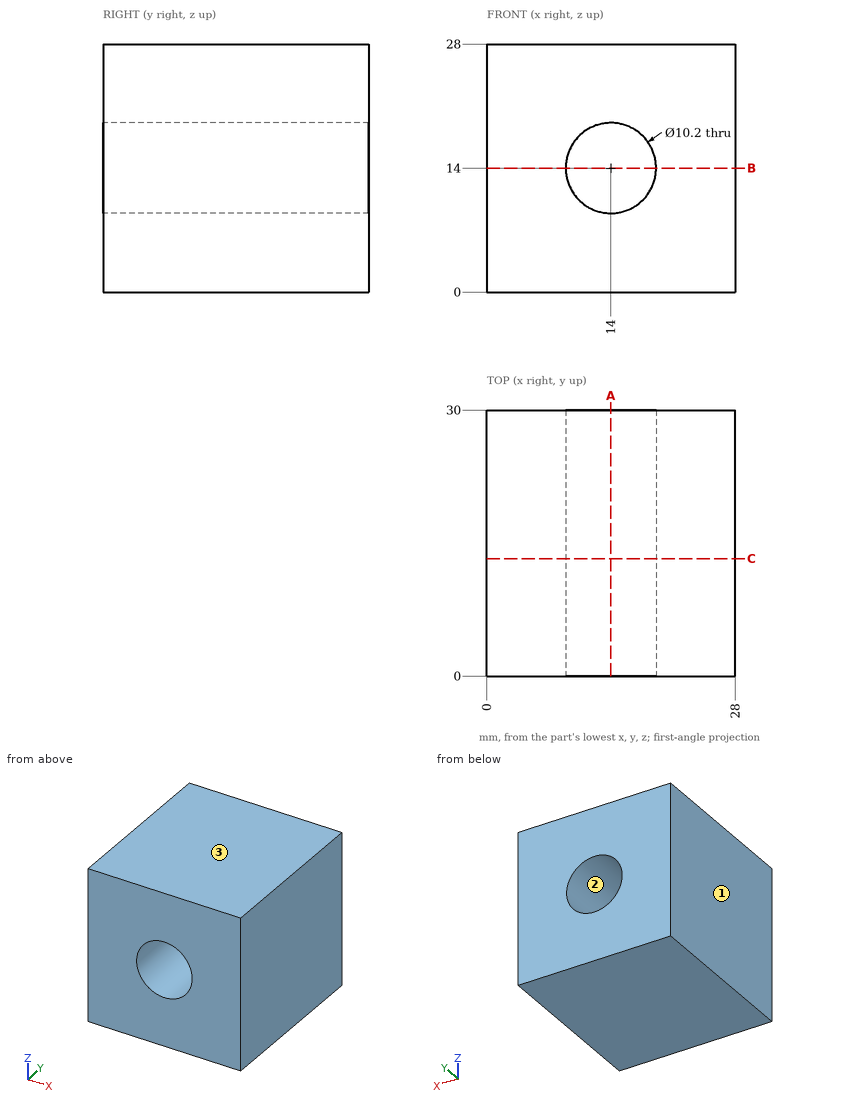
Input: dimensioned drawing with shaded views. Units: mm. Origin: part minimum x, y, z. Round coordinates to 2 decimals unless told otherwise and drop trailing zeros. Order: outer loops, then holes, each group sorted by start corner. A loop starts at its lowest first (then second) coordinate and runs counter-clockwise, first axis right, second up. Notation, with made-up numbers: (-30, 21.25) - (-7, 21.25) arc R34 ccw to (-7, 53.25) - close; hole circle Ø3 at (20.25, 82). An arc over 180 degrees is marked (long way). Write item = value, one per line. Start each with the question number.
Q1. Cut plane C-C on y = 13.25. Return the cut outline in (x, z), and give its area (3 significant figures).
Q2. Cut plane A-A on x = 14. Return the cut outline in (y, z), and give its area (3 significant figures).
Q3. Ray query, line 1 (Z direction, x = 14, y = 14.75); line 2 (Z direction, x = 17, y = 15); line 3 (X direction, y = 2.75, z = 11.5). Return the intervals inside material, ascending. Write a range as from..to.
Q4. Cut plane B-B on z = 14. Return the cut outline in (x, y), and give its area (3 significant figures).
Q5. Pull-direction query (X, two-part tool) for the marked faces 1, 2 and 3; classes: +X half, -X half, draft (parallel to the pull), parting line (faces both ways), or undercut.
Outcome:
q1.outline = (0, 0) - (28, 0) - (28, 28) - (0, 28) - close; hole circle Ø10.2 at (14, 14)
q1.area = 702 mm^2
q2.outline = (0, 0) - (30, 0) - (30, 8.9) - (0, 8.9) - close; (0, 19.1) - (30, 19.1) - (30, 28) - (0, 28) - close
q2.area = 534 mm^2
q3.line_1 = 0..8.9, 19.1..28
q3.line_2 = 0..9.88, 18.12..28
q3.line_3 = 0..9.55, 18.45..28
q4.outline = (0, 0) - (8.9, 0) - (8.9, 30) - (0, 30) - close; (19.1, 0) - (28, 0) - (28, 30) - (19.1, 30) - close
q4.area = 534 mm^2
q5.face_1 = -X half
q5.face_2 = undercut
q5.face_3 = draft
